from build123d import *

# Parameters (mm, degrees)
SKETCH1_W           = 23.896551724
SKETCH1_H           = 25.5
BOSS_EXTRUDE1_DEPTH = 30
CUT_EXTRUDE1_DEPTH  = 41.417912914
SKETCH4_W           = 10
SKETCH4_H           = 5
CUT_EXTRUDE3_DEPTH  = 41.417912914
SKETCH7_W           = 6
SKETCH7_H           = 20
CUT_EXTRUDE4_DEPTH  = 23.896551724
SKETCH9_W           = 23.896551724
SKETCH9_H           = 30
BOSS_EXTRUDE3_DEPTH = 17.5
SKETCH12_W          = 23.896551724
SKETCH12_H          = 30
CUT_EXTRUDE7_DEPTH  = 8
SKETCH15_W          = 23.896551724
SKETCH15_H          = 30
CUT_EXTRUDE11_DEPTH = 6
SKETCH18_W          = 23.896551724
SKETCH18_H          = 4
BOSS_EXTRUDE4_DEPTH = 7
SKETCH19_W          = 30
SKETCH19_H          = 5
CUT_EXTRUDE12_DEPTH = 44.140557302
SKETCH20_R          = 2.6
CUT_EXTRUDE13_DEPTH = 45.763392366
SKETCH21_W          = 23.896551724
SKETCH21_H          = 4
BOSS_EXTRUDE5_DEPTH = 5
SKETCH22_R          = 2.6
CUT_EXTRUDE14_DEPTH = 41.685670648
SKETCH23_R          = 6.5
CUT_EXTRUDE15_DEPTH = 3.2


with BuildPart() as part:
    # Sketch1 → Boss-Extrude1 (new body)
    with BuildSketch(Plane.XY):
        Rectangle(SKETCH1_W, SKETCH1_H)
    extrude(amount=BOSS_EXTRUDE1_DEPTH)

    # Sketch2 → Cut-Extrude1 (cut, through all)
    with BuildSketch(Plane(origin=(11.948275862, 0, 0), x_dir=(0, 0, -1), z_dir=(1, 0, 0))):
        Polygon((-15, -12.75), (-20, -12.75), (-20, 2.25), (-10, 2.25), (-10, -12.75), align=None)
    extrude(amount=-CUT_EXTRUDE1_DEPTH, mode=Mode.SUBTRACT)

    # Sketch4 → Cut-Extrude3 (cut, through all)
    with BuildSketch(Plane(origin=(11.948275862, 0, 0), x_dir=(0, 0, -1), z_dir=(1, 0, 0))):
        with Locations((-15, 4.75)):
            Rectangle(SKETCH4_W, SKETCH4_H)
    extrude(amount=-CUT_EXTRUDE3_DEPTH, mode=Mode.SUBTRACT)

    # Sketch7 → Cut-Extrude4 (cut)
    with BuildSketch(Plane.ZY.offset(11.948275862)):
        with Locations((7, -2.75)):
            Rectangle(SKETCH7_W, SKETCH7_H)
        with Locations((23, -2.75)):
            Rectangle(SKETCH7_W, SKETCH7_H)
    extrude(amount=-CUT_EXTRUDE4_DEPTH, mode=Mode.SUBTRACT)

    # Sketch9 → Boss-Extrude3 (add)
    with BuildSketch(Plane(origin=(0, 12.75, 0), x_dir=(1, 0, 0), z_dir=(0, 1, 0))):
        with Locations((0, -15)):
            Rectangle(SKETCH9_W, SKETCH9_H)
    extrude(amount=BOSS_EXTRUDE3_DEPTH)

    # Sketch12 → Cut-Extrude7 (cut)
    with BuildSketch(Plane(origin=(0, 30.25, 0), x_dir=(1, 0, 0), z_dir=(0, 1, 0))):
        with Locations((0, -15)):
            Rectangle(SKETCH12_W, SKETCH12_H)
    extrude(amount=-CUT_EXTRUDE7_DEPTH, mode=Mode.SUBTRACT)

    # Sketch15 → Cut-Extrude11 (cut)
    with BuildSketch(Plane(origin=(0, 22.25, 0), x_dir=(1, 0, 0), z_dir=(0, 1, 0))):
        with Locations((0, -15)):
            Rectangle(SKETCH15_W, SKETCH15_H)
    extrude(amount=-CUT_EXTRUDE11_DEPTH, mode=Mode.SUBTRACT)

    # Sketch18 → Boss-Extrude4 (add)
    with BuildSketch(Plane.XZ.offset(12.75)):
        with Locations((0, 28)):
            Rectangle(SKETCH18_W, SKETCH18_H)
        with Locations((0, 2)):
            Rectangle(SKETCH18_W, SKETCH18_H)
    extrude(amount=BOSS_EXTRUDE4_DEPTH)

    # Sketch19 → Cut-Extrude12 (cut, through all)
    with BuildSketch(Plane(origin=(11.948275862, 0, 0), x_dir=(0, 0, -1), z_dir=(1, 0, 0))):
        with Locations((-15, 13.75)):
            Rectangle(SKETCH19_W, SKETCH19_H)
    extrude(amount=-CUT_EXTRUDE12_DEPTH, mode=Mode.SUBTRACT)

    # Sketch20 → Cut-Extrude13 (cut, through all)
    with BuildSketch(Plane(origin=(0, 11.25, 0), x_dir=(1, 0, 0), z_dir=(0, 1, 0))):
        with Locations(Location((0, -15, 0), (0, 0, 270))):
            Circle(SKETCH20_R)
    extrude(amount=-CUT_EXTRUDE13_DEPTH, mode=Mode.SUBTRACT)

    # Sketch21 → Boss-Extrude5 (add)
    with BuildSketch(Plane.XZ.offset(19.75)):
        with Locations((0, 2)):
            Rectangle(SKETCH21_W, SKETCH21_H)
        with Locations((0, 28)):
            Rectangle(SKETCH21_W, SKETCH21_H)
    extrude(amount=BOSS_EXTRUDE5_DEPTH)

    # Sketch22 → Cut-Extrude14 (cut, through all)
    with BuildSketch(Plane.XY.offset(30)):
        with Locations((0, -14.25)):
            Circle(SKETCH22_R)
    extrude(amount=-CUT_EXTRUDE14_DEPTH, mode=Mode.SUBTRACT)

    # Sketch23 → Cut-Extrude15 (cut)
    with BuildSketch(Plane(origin=(0, 0, 0), x_dir=(-1, 0, 0), z_dir=(0, 0, -1))):
        with Locations((0, -14.25)):
            Circle(SKETCH23_R)
    cut_extrude15 = extrude(amount=-CUT_EXTRUDE15_DEPTH, mode=Mode.SUBTRACT)

    # Mirror1: Cut-Extrude15 across plane
    add(cut_extrude15.mirror(Plane(origin=(0, 0, 15), x_dir=(1, 0, 0), z_dir=(0, 0, -1))), mode=Mode.SUBTRACT)


solid = part.part
Can you work these out from the model? Positions are in its coordinate system, mm. A direction names the side the tool comes from. Give positions to 0.01 mm unless a question says otherwise; leave off trailing zeros. Loops run counter-clockwise (first coordinate to the right, second up) from the corner with the lowest first, then second, coordinate; pieces in that order, holes last. Notation, with made-up numbers: (-20.75, 47.5) - (8.25, 47.5) arc R8 ccw to (8.25, 62.5) - close; hole circle Ø5 at (-7.5, 80.5). An arc over 180 degrees is marked (long way). Answer as a JSON object with one key per item and string values.
Q1. Imagine slicing it at C-C on z = 15. Write out the boundary of the cut face in (x, y).
Geometry says:
{"outline": "(-11.95, 7.25) - (-2.6, 7.25) - (-2.6, 11.25) - (-11.95, 11.25) - close; (2.6, 7.25) - (11.95, 7.25) - (11.95, 11.25) - (2.6, 11.25) - close"}
Q2. Which directions (+Z, -Z, +X, -X, +Y, -Y) give clear straight access to the entire face, cutting with the end or side of a thin tool? Please do faces 1 (the flat face through (0, -9, 26)), 2 (the flat face through (3, 11.25, 15)), 3 (the flat face through (-3, -14, 3.2)), 4 (the flat face through (-3, -14, 26.8)).
Geometry says:
{"face 1": "+X, -X, -Y", "face 2": "+Z, -Z, +X, -X, +Y", "face 3": "-Z", "face 4": "+Z"}
Q3. Imagine slicing it at D-D on y = 6.5. Write out the boundary of the cut face in (x, z), plus the area to 3 significant figures.
Geometry says:
{"outline": "(-11.95, 0) - (11.95, 0) - (11.95, 4) - (-11.95, 4) - close; (-11.95, 26) - (11.95, 26) - (11.95, 30) - (-11.95, 30) - close", "area": "191 mm²"}
Q4. If I drill on L1, parallel to Z at x = -8.25, y = -4; L2, parallel to X at y = 9.1, z = 15; L3, parallel to Y at x = 0, z = 3.7, over which ranges is the centre line in solid material (lowest first)?
Geometry says:
{"L1": "0 to 4, 26 to 30", "L2": "-11.95 to -2.6, 2.6 to 11.95", "L3": "-24.75 to -16.85, -11.65 to 11.25"}
Q5. If we mould it in two halves opening along Y, with no side actions, what happens to faces 5 (the cylindrical face through (0.8, -7.8, 28.4)), 6 (the flat face through (0, 7.25, 12)), 7 (the flat face through (0, -6, 0)), 8 (the cylindrical face through (-0.56, -16.79, 26.41))? For each: pulls with the +Y half, pulls with the -Y half, needs draft (parallel to the pull), parting line crosses it, or undercut.
Geometry says:
{"face 5": "undercut", "face 6": "pulls with the -Y half", "face 7": "needs draft", "face 8": "undercut"}
Q6. Will these pins go through, and if not, where does the flat tip stop? P1, Ø11, axis at x = 2, z = 12, coming from the -Y side; P2, Ø8.5, axis at x = 0, y = -14.25, coming from the +Z side; P3, Ø5, axis at x = 9, y = -11.5, coming from the -Z side.
Geometry says:
{"P1": "y = 7.25", "P2": "z = 26.8", "P3": "z = 0"}
Q7. Imagine slicing it at A-A on y = -14.25. Write out the boundary of the cut face in (x, z), plus the area to 3 significant figures.
Geometry says:
{"outline": "(-11.95, 0) - (-6.5, 0) - (-6.5, 3.2) - (-2.6, 3.2) - (-2.6, 4) - (-11.95, 4) - close; (-11.95, 26) - (-2.6, 26) - (-2.6, 26.8) - (-6.5, 26.8) - (-6.5, 30) - (-11.95, 30) - close; (2.6, 3.2) - (6.5, 3.2) - (6.5, 0) - (11.95, 0) - (11.95, 4) - (2.6, 4) - close; (2.6, 26) - (11.95, 26) - (11.95, 30) - (6.5, 30) - (6.5, 26.8) - (2.6, 26.8) - close", "area": "99.7 mm²"}
Q8. Imagine slicing it at B-B on x = 0. Write out the boundary of the cut face in (y, z).
Geometry says:
{"outline": "(-24.75, 0) - (-20.75, 0) - (-20.75, 3.2) - (-16.85, 3.2) - (-16.85, 4) - (-24.75, 4) - close; (-24.75, 26) - (-16.85, 26) - (-16.85, 26.8) - (-20.75, 26.8) - (-20.75, 30) - (-24.75, 30) - close; (-11.65, 3.2) - (-7.75, 3.2) - (-7.75, 0) - (11.25, 0) - (11.25, 12.4) - (7.25, 12.4) - (7.25, 4) - (-11.65, 4) - close; (-11.65, 26) - (7.25, 26) - (7.25, 17.6) - (11.25, 17.6) - (11.25, 30) - (-7.75, 30) - (-7.75, 26.8) - (-11.65, 26.8) - close"}
